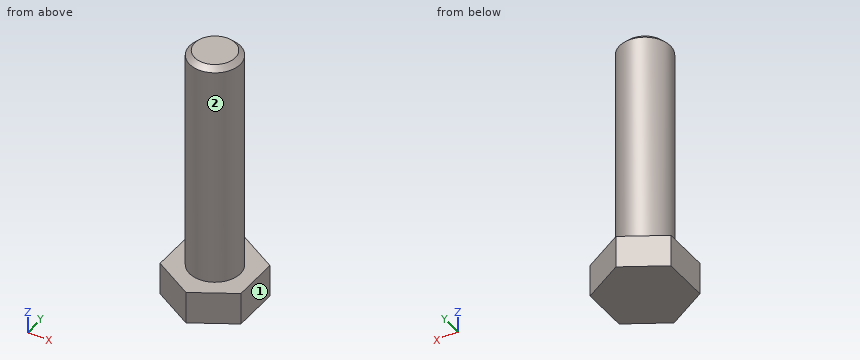
from build123d import *

# Parameters (mm, degrees)
BOSS_EXTRUDE1_DEPTH = 6.4
SKETCH3_R           = 5
BOSS_EXTRUDE2_DEPTH = 45
CHAMFER1_SIZE       = 1


with BuildPart() as part:
    # Sketch1 → Boss-Extrude1 (new body)
    with BuildSketch(Plane.XY):
        Polygon((8, 4.618802154), (0, 9.237604307), (-8, 4.618802154), (-8, -4.618802154), (0, -9.237604307), (8, -4.618802154), align=None)
    extrude(amount=BOSS_EXTRUDE1_DEPTH)

    # Sketch3 → Boss-Extrude2 (add)
    with BuildSketch(Plane.XY.offset(6.4)):
        with Locations(Location((0, 0, 0), (0, 0, 180))):
            Circle(SKETCH3_R)
    extrude(amount=BOSS_EXTRUDE2_DEPTH)

    # Chamfer1
    chamfer1_edges = [part.edges().sort_by_distance(p)[0] for p in [
        (5, 0, 51.4),
    ]]
    chamfer(chamfer1_edges, length=CHAMFER1_SIZE)


solid = part.part
The listing builds one solid part. Answer for the finished solid, in the listing's coordinates (mm). Face numbers are marked on the shaded views. A direction names the side the tool comes from. Round coordinates to 2 decimals unless told otherwise and drop trailing zeros. Order: outer loops, then holes, each group sorted by start corner. A loop starts at its lowest first (then second) coordinate and runs counter-clockwise, first axis right, second up. Notation, with made-up numbers: (64, 56.25) -> (84, 56.25) arc R21 ccw to (84, 73.25) -> close; hole circle Ø4 at (11.5, 70.25). An arc over 180 degrees is marked (long way). Write each question's results on one line, items separated by ' | '. Start each with the question number.
Q1. Each of these flat-tipped pins is pushed along its axis until it touches: pin 1 (3 mm diameter, centred on x = 0.5, y = -6, fed in from +Z); pin 2 (6 mm diameter, centred on x = -5, z = 19.5, fed in from -Y); pin 3 (5 mm diameter, centred on y = -6, z = 10, fed in from +X). Where does it stop, or does it pass through?
Q2. Find section C-C (z = 20.5). Determine the outline of the cut face in (x, y).
Q3. Find section B-B (z = 5). Determine the outline of the cut face in (x, y), then the cut area to 3 significant figures.
Q4. Which of the six approach directions +Z, -Z, +X, -X, +Y, -Y give full straight-line access (tool end or side, diameter ignored) to the marked faces 1 and 2?
Q5. Find section A-A (y = 0). Determine the outline of the cut face in (x, z).
Q6. Find section D-D (y = -5.5). Determine the outline of the cut face in (x, z).
Q7. Straight lines are drawn through the part: probe 1 along Z at (x, y) = (5.75, 0.25); probe 2 along Y at (x, z) = (-2, 41.5); probe 3 along Y at (x, z) = (1.5, 22). For each, find the intervals that lie inside material, in ascending order. Write a range as from..to.
Worked answers:
1) pin 1: stops at z = 50.88 | pin 2: stops at y = -4.58 | pin 3: stops at x = 3.57
2) outline: circle Ø10 at (0, 0)
3) outline: (-8, -4.62) -> (0, -9.24) -> (8, -4.62) -> (8, 4.62) -> (0, 9.24) -> (-8, 4.62) -> close | area: 222 mm2
4) face 1: +Z, -Z, +X, +Y, -Y | face 2: +Z
5) outline: (-8, 0) -> (8, 0) -> (8, 6.4) -> (5, 6.4) -> (5, 50.4) -> (4, 51.4) -> (-4, 51.4) -> (-5, 50.4) -> (-5, 6.4) -> (-8, 6.4) -> close
6) outline: (-6.47, 0) -> (6.47, 0) -> (6.47, 6.4) -> (-6.47, 6.4) -> close
7) probe 1: z = 0..6.4 | probe 2: y = -4.58..4.58 | probe 3: y = -4.77..4.77
